The drawing under review shows one solid part. Ordinate dimensions are in mm from its lowest x, y, z. A direction names the side the tool comes from. Coordinates: 2 decimals unless noted, no trailing zeros. Order: outer loops, then holes, each group sorted by start corner. A loop starts at its lowest first (then second) coordinate and runs counter-clockwise, first axis right, second up. Notation, with made-up numbers: (55.25, 48) -> (92.25, 48) arc R17 ccw to (92.25, 60) -> close; hole circle Ø6 at (88.5, -20). An arc over 180 degrees is marked (long way). Write item = value, one per line.
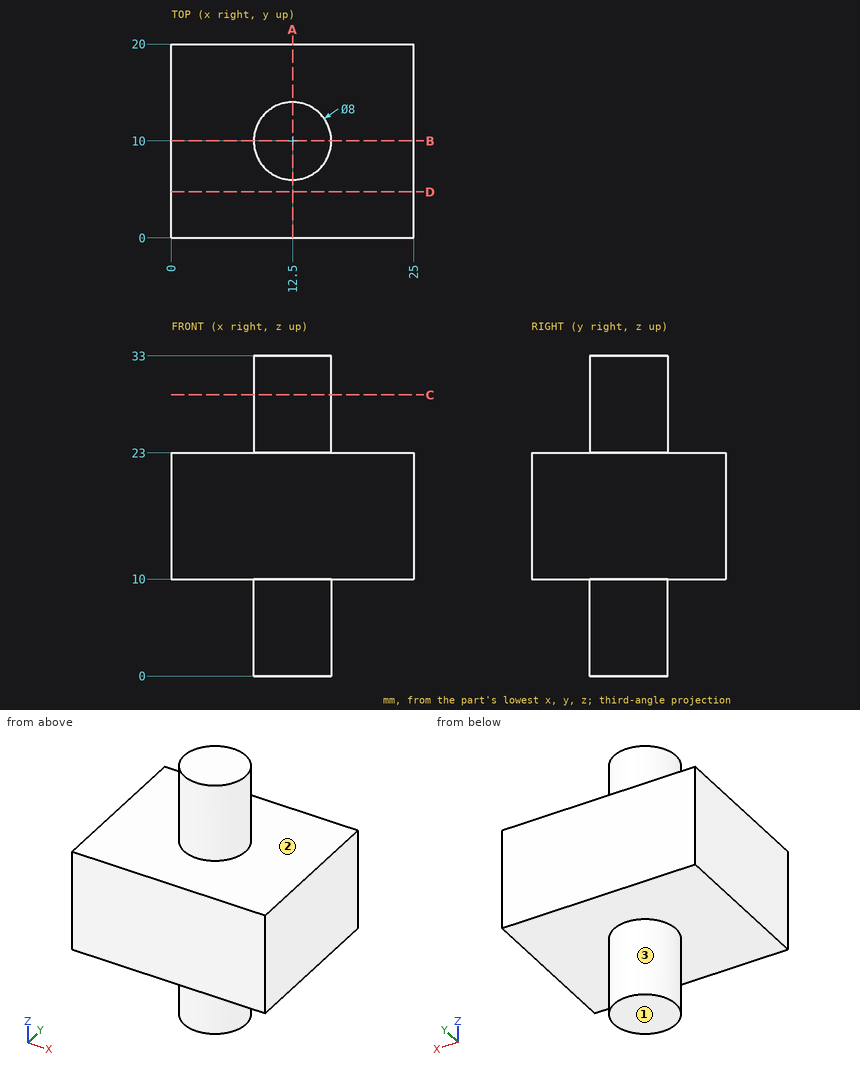
(1) Insertion check: pin 1 (8 mm diameter, centred on x = 20.5, y = 7, fed in from -Z); pin 2 (8 mm diameter, centred on x = 4, y = 10.5, fed in from +Z). Each pin has a flat end and moves straight along its axis. Give the tip position at first contact, or say it passes through.
Report:
pin_1 = 10
pin_2 = 23
(2) We need section A-A (x = 12.5). Write out the cut boundary in (y, z).
Report:
outline = (0, 10) -> (6, 10) -> (6, 0) -> (14, 0) -> (14, 10) -> (20, 10) -> (20, 23) -> (14, 23) -> (14, 33) -> (6, 33) -> (6, 23) -> (0, 23) -> close
(3) For L1, parallel to Z at x = 19.25, y = 17; L2, parallel to Y at x = 12.25, z = 23.5; L3, parallel to Y at x = 9, z = 24.5, list the stretches that pass through material, from the lowest coordinate up.
Report:
L1 = 10 to 23
L2 = 6.01 to 13.99
L3 = 8.06 to 11.94
(4) We need section B-B (y = 10). Write out the cut boundary in (x, z).
Report:
outline = (0, 10) -> (8.5, 10) -> (8.5, 0) -> (16.5, 0) -> (16.5, 10) -> (25, 10) -> (25, 23) -> (16.5, 23) -> (16.5, 33) -> (8.5, 33) -> (8.5, 23) -> (0, 23) -> close
(5) We need section D-D (y = 4.75). Write out the cut boundary in (x, z).
Report:
outline = (0, 10) -> (25, 10) -> (25, 23) -> (0, 23) -> close
(6) We need section C-C (z = 29). Write out the cut boundary in (x, y), and give its area (3 significant figures).
Report:
outline = circle Ø8 at (12.5, 10)
area = 50.3 mm²
(7) For the marked faces 1, 2 and 3, list the 3-axis set-ups (+Z, -Z, +X, -X, +Y, -Y) from which the entire face can be reached by the end or side of a thin tool; tool diameter is ignored.
Report:
face_1 = -Z, +X, -X, +Y, -Y
face_2 = +Z
face_3 = -Z
